Input: dimensioned drawing with shaded views. Units: mm. Origin: part minimum x, y, z. Give positions to 0.01 mm unless a question says otherwise; leave off trailing zeros. Write each loop counter-clockwise with the first axis right and the second up, starting at its lowest first coordinate (ties: lowest second). Pieces come first, ordered by that corner, then holes.
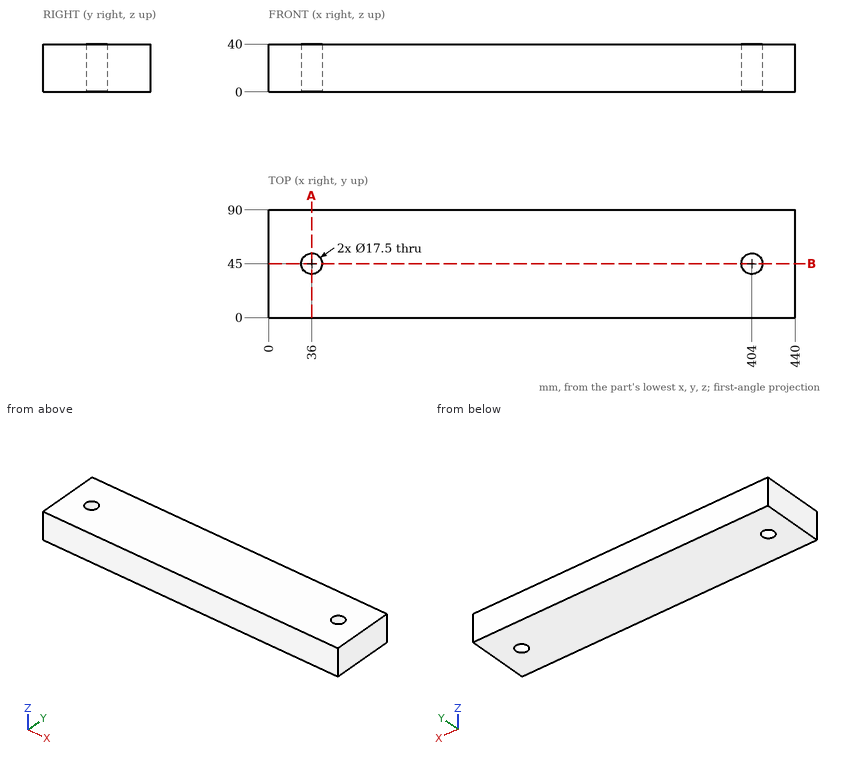
Item 1: Section A-A, the plane x = 36. Return the cut outline in (y, z).
Found:
outline: (0, 0) - (36.25, 0) - (36.25, 40) - (0, 40) - close; (53.75, 0) - (90, 0) - (90, 40) - (53.75, 40) - close
Item 2: Section B-B, the plane y = 45. Return the cut outline in (x, z), plus the area to 3 significant figures.
Found:
outline: (0, 0) - (27.25, 0) - (27.25, 40) - (0, 40) - close; (44.75, 0) - (395.25, 0) - (395.25, 40) - (44.75, 40) - close; (412.75, 0) - (440, 0) - (440, 40) - (412.75, 40) - close
area: 16,200 mm2
Item 3: Pin query (flat end, axial travel): pin 1 Ø10.5 at (x, y) = (36, 45) entering from +Z. Return the tip coordinate at first contact, or that it passes through.
Found:
pin 1: passes through
Item 4: Line query: L1, parallel to X at y = 46, z = 30; L2, parallel to Y at x = 404, z = 25; L3, parallel to X at y = 46.5, z = 30. Output: solid intervals per line, ascending.
Found:
L1: x = 0 to 27.31, 44.69 to 395.31, 412.69 to 440
L2: y = 0 to 36.25, 53.75 to 90
L3: x = 0 to 27.38, 44.62 to 395.38, 412.62 to 440
